The model under review builds one solid part; all positions refer to its coordinate system, in mm. A direction names the side the tool comes from. Coordinates: 2 decimals unless noted, no trailing zeros. Order: outer loops, then holes, each group sorted by start corner. A loop starts at its lowest first (then second) coordinate and runs counter-clockwise, first axis right, second up. Notation, with made-up numbers: M -29,45 L -15,45 A27 cw -15,71 Z; hole C 85.25,83.25 d6. An arc over 180 degrees is marked long. Answer as CSV lines item,"result". Start each with the question number.
Q1. Wall thickness on L1, parallel to Z at x = 5.5, y = 2; L2, parallel to X at y = -0.5, z = -52; L3, parallel to Z at x = -5, y = 13: over which ranges is each line inside the solid? List them lowest first. Write a range as [from, to].
Q2. For P1, Ø4, axis at x = -8.5, z = -60, coming from the +Y side; P2, Ø8.5, axis at x = 1, y = 4.5, coming from the -Z side; P3, Ø4, axis at y = 12, z = -45, coming from the -X side; P4, Ø5, axis at x = -4, z = -49, coming from the +Y side, all flat-tipped, find the tip position at first contact; note any pin that passes through.
Q3. Consider section A-A on y = 0. Write out the cut boundary in (x, z).
Q4. Consider section C-C on z = -21. Write out the cut boundary in (x, y).
Q5. Machinability: for faces 1 (the face through (0, 0, 0)), 2 (the face through (-10, 0, -6)), 3 (the face through (-2, 5, -73.5)), which of the approach directions +Z, -Z, +X, -X, +Y, -Y give a long, thin tool a straight path to every point of the face, cutting with its end or side? Answer none if there is none.
from build123d import *

# Parameters (mm, degrees)
CHAMFER1_SIZE = 0.5


with BuildPart() as part:
    # Sketch1 → Revolve1 (revolve)
    with BuildSketch(Plane(origin=(0, 0, 0), x_dir=(0, 0, -1), z_dir=(1, 0, 0)), mode=Mode.PRIVATE) as revolve1_sk:
        Polygon((81.5, 0), (81.5, 5.05), (73.5, 5.05), (73.5, 7.5), (70, 7.5), (70, 15), (11, 15), (11, 10), (0, 10), (0, 0), align=None)
    revolve(revolve1_sk.sketch.rotate(Axis((0, 0, 0), (0, 0, -1)), 90), axis=Axis((0, 0, 0), (0, 0, -1)))

    # Chamfer1
    chamfer1_edges = [part.edges().sort_by_distance(p)[0] for p in [
        (-7.5, 0, -73.5),
        (-5.05, 0, -81.5),
        (-10, 0, 0),
        (-15, 0, -11),
        (-15, 0, -70),
    ]]
    chamfer(chamfer1_edges, length=CHAMFER1_SIZE)


solid = part.part
Evaluation:
1,L1,"z = [-73.5, 0]"
1,L2,"x = [-14.99, 14.99]"
1,L3,"z = [-70, -11]"
2,P1,"stops at y = 13.52"
2,P2,"stops at z = -81.5"
2,P3,"stops at x = -11.18"
2,P4,"stops at y = 14.92"
3,outline,"M -15,-69.5 L -14.5,-70 L -7.5,-70 L -7.5,-73 L -7,-73.5 L -5.05,-73.5 L -5.05,-81 L -4.55,-81.5 L 4.55,-81.5 L 5.05,-81 L 5.05,-73.5 L 7,-73.5 L 7.5,-73 L 7.5,-70 L 14.5,-70 L 15,-69.5 L 15,-11.5 L 14.5,-11 L 10,-11 L 10,-0.5 L 9.5,0 L -9.5,0 L -10,-0.5 L -10,-11 L -14.5,-11 L -15,-11.5 Z"
4,outline,"C 0,0 d30"
5,face 1,"+Z, +X, -X, +Y, -Y"
5,face 2,"+Z"
5,face 3,"-Z"
